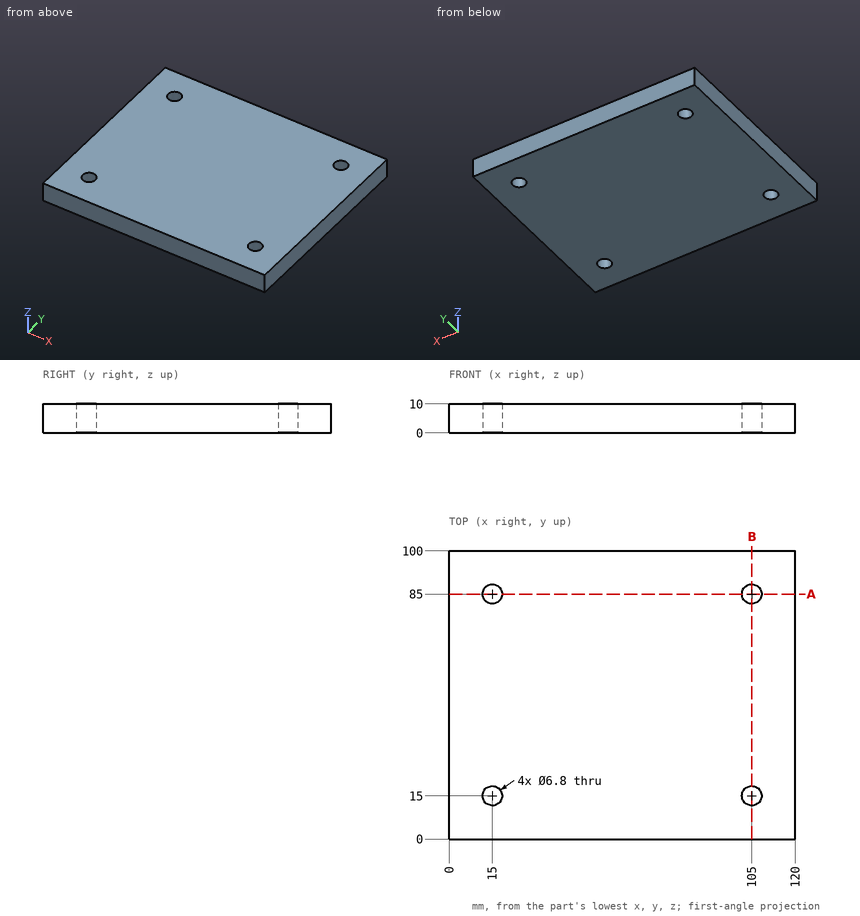
Verification items for this drawing (mm, ordinates from the low corner). Give positions to 0.01 mm unless a question says otherwise; leave off trailing zeros. Loops run counter-clockwise (first coordinate to the right, second up) from the corner with the lowest first, then second, coordinate; pieces in that order, holes last. Notation, with made-up numbers: M 84,67.25 L 116,67.25 A23 cw 116,101.25 Z; hole C -31.75,62 d2. An arc over 180 degrees is marked long. Answer as a JSON object with one key per item and string values. Group by question number.
Item 1: Sectioned sample at B-B on x = 105. Record the boundary of the cut face in (y, z).
Item 2: Sectioned sample at A-A on y = 85. Record the boundary of the cut face in (x, z), plus the area to 3 significant figures.
Item 3: Material ranges on L1, parallel to Y at x = 15, z = 7.25; L2, parallel to Y at x = 13, z = 5.5, recorded low to high.
Item 4: Gauge pin test, flat end, axial feed: pin 1 (5.5 mm diameter, centred on x = 15, y = 85, fed in from +Z). Record the tip position at first contact, or that the pin passes through.
Findings below:
{
 "1": {"outline": "M 0,0 L 11.6,0 L 11.6,10 L 0,10 Z; M 18.4,0 L 81.6,0 L 81.6,10 L 18.4,10 Z; M 88.4,0 L 100,0 L 100,10 L 88.4,10 Z"},
 "2": {"outline": "M 0,0 L 11.6,0 L 11.6,10 L 0,10 Z; M 18.4,0 L 101.6,0 L 101.6,10 L 18.4,10 Z; M 108.4,0 L 120,0 L 120,10 L 108.4,10 Z", "area": "1,060 mm2"},
 "3": {"L1": "0 to 11.6, 18.4 to 81.6, 88.4 to 100", "L2": "0 to 12.25, 17.75 to 82.25, 87.75 to 100"},
 "4": {"pin 1": "through"}
}
